The listing builds one solid part. Answer for the finished solid, in the listing's coordinates (mm). Round coordinates to 2 decimals unless told otherwise and drop trailing zeros. Order: outer loops, then holes, each group sorted by start corner. A loop starts at its lowest first (then second) coordinate and runs counter-clockwise, first axis right, second up. Notation, with made-up numbers: (38, -22) - (60, -22) arc R11 cw to (60, -8) - close; hole circle Ø4 at (-35, 9.25). An arc over 180 degrees is marked (long way). One line per item, written item: value. Start each with the question number.
1. Straight lines are drawn through the part: line 1 (Y direction, x = 12, z = 0); line 2 (X direction, y = 3.5, z = 1.25); line 3 (Y direction, x = 19.5, z = 1). For each, find the intervals that lie inside material, in ascending order.
2. Flat-ended cylindrical pins translate along their axes: P1, Ø1, axis at x = 15, z = 3, coming from the +Y side; P2, Ø1, axis at x = 7.5, z = -1.5, coming from the +Y side; P3, Ø3, axis at x = 21.5, y = 1.5, coming from the -Z side; P4, Ø4, axis at x = 7, z = -2.5, coming from the -Y side. Find the tip coordinate at first contact, or state that the pin passes through.
3. Section A-A, the plane x = 1.5 is taken. Give the vertices of the cut face in (y, z), then the cut area to 3 significant figures.
from build123d import *

# Parameters (mm, degrees)
PATTERN_LINEAR_1_COUNT   = 30
PATTERN_LINEAR_1_PITCH   = 0.7
PATTERN_CIRCULAR_1_COUNT = 2
PATTERN_CIRCULAR_1_ANGLE = 90


with BuildPart() as part:
    # 草图1 → Revolve 689 (revolve)
    with BuildSketch(Plane.XY, mode=Mode.PRIVATE) as revolve_689_sk:
        with BuildLine():
            Line((0, 0), (0, 4.2))
            Line((0, 4.2), (0.232, 4.2))
            Line((0.232, 4.2), (2.407106781, 2.024893219))
            ThreePointArc((2.407106781, 2.024893219), (2.73153013, 1.808120467), (3.114213562, 1.732))
            Line((3.114213562, 1.732), (3.635810384, 1.732))
            Line((3.635810384, 1.732), (4.1, 2))
            Line((4.1, 2), (25, 2))
            Line((25, 2), (25, 0))
            Line((25, 0), (0, 0))
        make_face()
    revolve(revolve_689_sk.sketch.rotate(Axis((0, 0, 0), (1, 0, 0)), 90), axis=Axis((0, 0, 0), (1, 0, 0)))

    # 草图2 → 切除-旋转1 (revolve, cut)
    with BuildSketch(Plane.XY, mode=Mode.PRIVATE) as cut_revolve_1_sk:
        Polygon((24.653791204, 2), (25.353791204, 2), (25, 1.3938), align=None)
    cut_revolve_1 = revolve(cut_revolve_1_sk.sketch.rotate(Axis((0, 0, 0), (-1, 0, 0)), 270), axis=Axis((0, 0, 0), (-1, 0, 0)), mode=Mode.SUBTRACT)

    # 阵列(线性)1: 切除-旋转1 ×30
    with Locations(*[(-i * PATTERN_LINEAR_1_PITCH, 0, 0) for i in range(1, PATTERN_LINEAR_1_COUNT)]):
        add(cut_revolve_1, mode=Mode.SUBTRACT)

    # 草图3 → 切除-放样1 section 0
    with BuildSketch(Plane.ZY, mode=Mode.PRIVATE) as loft_1_s0:
        with BuildLine():
            Line((-2.3, 0.35), (2.3, 0.35))
            Line((2.3, 0.35), (2.3, -0.35))
            Line((2.3, -0.35), (-2.3, -0.35))
            Line((-2.3, -0.35), (-2.3, 0.35))
        make_face()
    loft_1 = loft([loft_1_s0.sketch, Vertex(2.6, 0, 0)], mode=Mode.SUBTRACT)

    # 阵列(圆周)1: 切除-放样1 ×2 about axis
    pattern_circular_1_axis = Axis((0, 0, 0), (1, 0, 0))
    for i in range(1, PATTERN_CIRCULAR_1_COUNT):
        add(loft_1.rotate(pattern_circular_1_axis, i * PATTERN_CIRCULAR_1_ANGLE / (PATTERN_CIRCULAR_1_COUNT - 1)), mode=Mode.SUBTRACT)


solid = part.part
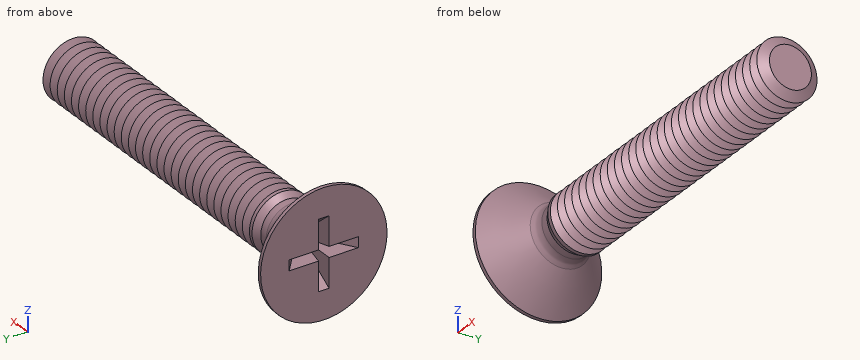
Answer list:
1. line 1: y = -1.91 to 1.91
1. line 2: x = 0 to 0.72
1. line 3: y = -1.2 to 1.2
2. P1: passes through
2. P2: stops at y = 1.64
2. P3: stops at z = -2
2. P4: stops at y = -1.93
3. outline: circle Ø5.86 at (0, 0); hole (-0.97, -0.15) - (-0.15, -0.15) - (-0.15, -0.97) - (0.15, -0.97) - (0.15, -0.15) - (0.97, -0.15) - (0.97, 0.15) - (0.15, 0.15) - (0.15, 0.97) - (-0.15, 0.97) - (-0.15, 0.15) - (-0.97, 0.15) - close
3. area: 25.9 mm²
